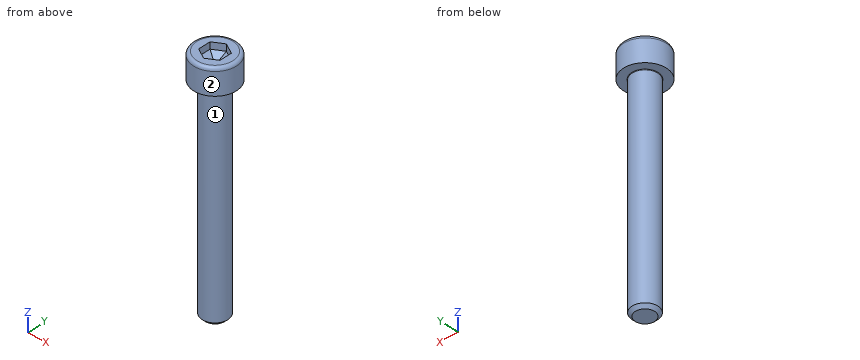
from build123d import *
from OCP.BRepFilletAPI import BRepFilletAPI_MakeChamfer

# Parameters (mm, degrees)
SKETCH1_R           = 5
BOSS_EXTRUDE1_DEPTH = 6
CUT_EXTRUDE1_DEPTH  = 3
SKETCH3_R           = 3
BOSS_EXTRUDE2_DEPTH = 50
CHAMFER1_SIZE       = 0.75
FILLET1_R           = 0.769230769
CHAMFER2_SIZE       = 1.44092219
CHAMFER2_SIZE2      = 2.495750443
FILLET2_R           = 0.1


with BuildPart() as part:
    # Sketch1 → Boss-Extrude1 (new body)
    with BuildSketch(Plane.XY):
        Circle(SKETCH1_R)
    extrude(amount=BOSS_EXTRUDE1_DEPTH)

    # Sketch2 → Cut-Extrude1 (cut)
    with BuildSketch(Plane.XY.offset(6)):
        Polygon((2.5, 1.443375673), (0, 2.886751346), (-2.5, 1.443375673), (-2.5, -1.443375673), (0, -2.886751346), (2.5, -1.443375673), align=None)
    extrude(amount=-CUT_EXTRUDE1_DEPTH, mode=Mode.SUBTRACT)

    # Sketch3 → Boss-Extrude2 (add)
    with BuildSketch(Plane(origin=(0, 0, 0), x_dir=(-1, 0, 0), z_dir=(0, 0, -1))):
        with Locations(Location((0, 0, 0), (0, 0, 180))):
            Circle(SKETCH3_R)
    extrude(amount=BOSS_EXTRUDE2_DEPTH)

    # Chamfer1
    chamfer1_edges = [part.edges().sort_by_distance(p)[0] for p in [
        (-3, 0, -50),
    ]]
    chamfer(chamfer1_edges, length=CHAMFER1_SIZE)

    # Fillet1
    fillet1_edges = [part.edges().sort_by_distance(p)[0] for p in [
        (-5, 0, 6),
    ]]
    fillet(fillet1_edges, radius=FILLET1_R)

    # Chamfer2: one chamfer whose edges measure the first distance from different faces: ONE call of the kernel's chamfer builder (chamfer() names one face for all edges)
    chamfer2_edges_1 = [part.edges().sort_by_distance(p)[0] for p in [
        (-1.25, 2.165063509, 3),
    ]]
    chamfer2_side_1 = [part.faces().sort_by_distance(p)[0] for p in [
        (-1.25, 2.165063509, 4.5),
    ]]
    chamfer2_edges_2 = [part.edges().sort_by_distance(p)[0] for p in [
        (1.25, 2.165063509, 3),
    ]]
    chamfer2_side_2 = [part.faces().sort_by_distance(p)[0] for p in [
        (1.25, 2.165063509, 4.5),
    ]]
    chamfer2_edges_3 = [part.edges().sort_by_distance(p)[0] for p in [
        (2.5, 0, 3),
    ]]
    chamfer2_side_3 = [part.faces().sort_by_distance(p)[0] for p in [
        (2.5, 0, 4.5),
    ]]
    chamfer2_edges_4 = [part.edges().sort_by_distance(p)[0] for p in [
        (1.25, -2.165063509, 3),
    ]]
    chamfer2_side_4 = [part.faces().sort_by_distance(p)[0] for p in [
        (1.25, -2.165063509, 4.5),
    ]]
    chamfer2_edges_5 = [part.edges().sort_by_distance(p)[0] for p in [
        (-1.25, -2.165063509, 3),
    ]]
    chamfer2_side_5 = [part.faces().sort_by_distance(p)[0] for p in [
        (-1.25, -2.165063509, 4.5),
    ]]
    chamfer2_edges_6 = [part.edges().sort_by_distance(p)[0] for p in [
        (-2.5, 0, 3),
    ]]
    chamfer2_side_6 = [part.faces().sort_by_distance(p)[0] for p in [
        (-2.5, 0, 4.5),
    ]]
    chamfer2 = BRepFilletAPI_MakeChamfer(part.part.solid().wrapped)
    for e in chamfer2_edges_1:
        chamfer2.Add(CHAMFER2_SIZE, CHAMFER2_SIZE2, e.wrapped, chamfer2_side_1[0].wrapped)  # the first distance lies on this face
    for e in chamfer2_edges_2:
        chamfer2.Add(CHAMFER2_SIZE, CHAMFER2_SIZE2, e.wrapped, chamfer2_side_2[0].wrapped)  # the first distance lies on this face
    for e in chamfer2_edges_3:
        chamfer2.Add(CHAMFER2_SIZE, CHAMFER2_SIZE2, e.wrapped, chamfer2_side_3[0].wrapped)  # the first distance lies on this face
    for e in chamfer2_edges_4:
        chamfer2.Add(CHAMFER2_SIZE, CHAMFER2_SIZE2, e.wrapped, chamfer2_side_4[0].wrapped)  # the first distance lies on this face
    for e in chamfer2_edges_5:
        chamfer2.Add(CHAMFER2_SIZE, CHAMFER2_SIZE2, e.wrapped, chamfer2_side_5[0].wrapped)  # the first distance lies on this face
    for e in chamfer2_edges_6:
        chamfer2.Add(CHAMFER2_SIZE, CHAMFER2_SIZE2, e.wrapped, chamfer2_side_6[0].wrapped)  # the first distance lies on this face
    add(Compound.cast(chamfer2.Shape()), mode=Mode.REPLACE)

    # Fillet2
    fillet2_edges = [part.edges().sort_by_distance(p)[0] for p in [
        (-3, 0, 0),
    ]]
    fillet(fillet2_edges, radius=FILLET2_R)


solid = part.part
Here's how the part is built. I have some questions about the finished solid (model axes, mm). Face numbers are marked on the shaded views. A direction names the side the tool comes from. Give positions to 0.01 mm unless a question says otherwise; leave off trailing zeros. Order: outer loops, then holes, each group sorted by start corner. A loop starts at its lowest first (then second) coordinate and runs counter-clockwise, first axis right, second up. Notation, with made-up numbers: (3, 70) -> (17, 70) arc R18 ccw to (17, 102) -> close; hole circle Ø6 at (-24.75, -36). An arc over 180 degrees is marked (long way). One line per item, written item: value. Start each with the question number.
1. I need wall thicknesses on probe 1 along Z at (x, y) = (-3, 1.5); probe 2 along Z at (x, y) = (-1, -2.5); probe 3 along Y at (x, z) = (0, -21). Which ranges of each line are inside material? Lowest first, please. Write a range as from..to.
2. Imagine slicing it at A-A, the plane z = -31.5. List the corners of the cut face in (x, y) for me.
3. Will these pins go through, and if not, where does the flat tip stop? pin 1 Ø5 at (x, z) = (2, -26.5) entering from +Y; pin 2 Ø3 at (y, z) = (-2.5, -3) entering from -X; pin 3 Ø6 at (x, z) = (3, -7.5) entering from -Y.
4. For the marked faces 1 and 2, which set-ups out of +Z, -Z, +X, -X, +Y, -Y let a thin tool reach every point of the face, with its end or its side?
Values follow:
1. probe 1: z = 0..6
1. probe 2: z = -49.56..6
1. probe 3: y = -3..3
2. outline: circle Ø6 at (0, 0)
3. pin 1: stops at y = 3
3. pin 2: stops at x = -2.83
3. pin 3: stops at y = -3
4. face 1: -Z
4. face 2: +Z, -Z
